Drawing for the job (mm, zero at the part's lowest x, y, z). Give positions to 0.01 mm unless a question says otherwise; leave off trailing zeros. Loops run counter-clockwise (first coordinate to the right, second up) from the corner with the lowest first, then second, coordinate; pieces in that order, holes last. Notation, with made-up numbers: M 40,76.5 L 48,76.5 A9 ccw 48,85.5 Z; hole C 6.25,50 d5. An arc over 180 degrees is marked long. Answer in a Markdown table with one row per item. Add a question column.
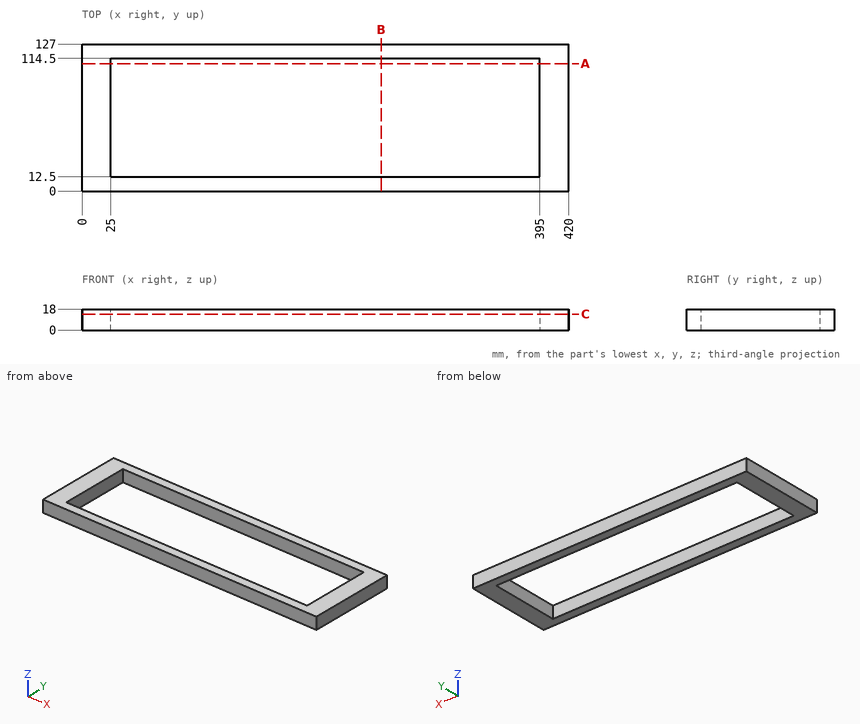
(1) Slice it at C-C, the plane z = 13.75. Give the cut face in (x, y), then the cut area to 3 significant figures.
(2) Slice it at A-A, the plane y = 110. Give the cut face in (x, z).
(3) Wall check: line 1 (Y direction, x = 180.5, z = 13.25); line 2 (X direction, y = 30, z = 9.5). Give the ranges that are in metal, low to high.
(4) Slice it at B-B, the plane x = 258. Give the cut face in (y, z).
Solution:
| question | item | result |
|---|---|---|
| 1 | outline | M 0,0 L 420,0 L 420,127 L 0,127 Z; hole M 25,12.5 L 395,12.5 L 395,114.5 L 25,114.5 Z |
| 1 | area | 15,600 mm^2 |
| 2 | outline | M 0,0 L 25,0 L 25,18 L 0,18 Z; M 395,0 L 420,0 L 420,18 L 395,18 Z |
| 3 | line 1 | 0 to 12.5, 114.5 to 127 |
| 3 | line 2 | 0 to 25, 395 to 420 |
| 4 | outline | M 0,0 L 12.5,0 L 12.5,18 L 0,18 Z; M 114.5,0 L 127,0 L 127,18 L 114.5,18 Z |
